Work out the finished part from the listing and answer in its coordinate system (mm). Coordinates: 2 decimals unless noted, no trailing zeros. Loops run counter-clockwise (first coordinate to the right, second up) from the corner with the lowest first, then second, coordinate; pieces in that order, holes last. Notation, with made-up numbers: (88.25, -8.75) -> (145.25, -8.75) arc R18 ccw to (145.25, 9.25) -> close; hole circle Ø9 at (-38.75, 82.5). An arc over 180 degrees is marked (long way). Use a Markdown table: item, result.
from build123d import *

# Parameters (mm, degrees)
SKETCH_1_R          = 38
EXTRUDE_1_DEPTH     = 678
SKETCH_2_R          = 7.5
EXTRUDE_2_DEPTH     = 146.75
SKETCH_3_R          = 8.25
EXTRUDE_4_DEPTH     = 76
EXTRUDE_START       = 76
SKETCH_4_R          = 8.25
EXTRUDE_5_DEPTH     = 76
CUT_EXTRUDE_START   = 7.5
CUT_EXTRUDE_2_DEPTH = 3
SKETCH_9_R          = 14.996083322
CUT_EXTRUDE_4_DEPTH = 34.45


with BuildPart() as part:
    # 草图1 → 凸台-拉伸1 (new, symmetric)
    with BuildSketch(Plane.XY):
        Circle(SKETCH_1_R)
    extrude(amount=EXTRUDE_1_DEPTH, both=True)

    # 草图2 → 凸台-拉伸2 (add, symmetric)
    with BuildSketch(Plane.XY.offset(678)):
        with Locations(Location((0, 0, 0), (0, 0, 180))):
            Circle(SKETCH_2_R)
    extrude_2 = extrude(amount=EXTRUDE_2_DEPTH, both=True)

    # 镜向1: 凸台-拉伸2 across plane
    add(extrude_2.mirror(Plane.XY))

    # 草图3 → 凸台-拉伸4 (add)
    with BuildSketch(Plane.XY.offset(678)):
        Circle(SKETCH_3_R)
    extrude(amount=EXTRUDE_4_DEPTH)

    # 草图4 → 凸台-拉伸5 (add)
    with BuildSketch(Plane(origin=(0, 0, -678), x_dir=(-1, 0, 0), z_dir=(0, 0, -1)).offset(EXTRUDE_START)):
        with Locations(Location((0, 0, 0), (0, 0, 180))):
            Circle(SKETCH_4_R)
    extrude(amount=-EXTRUDE_5_DEPTH)

    # 草图6 → 切除-拉伸2 (cut)
    with BuildSketch(Plane(origin=(0, 0, 0), x_dir=(1, 0, 0), z_dir=(0, 1, 0)).offset(CUT_EXTRUDE_START)):
        with BuildLine():
            Line((-2.5, -824.75), (-2.5, -809.75))
            ThreePointArc((-2.5, -809.75), (0, -807.25), (2.5, -809.75))
            Line((2.5, -809.75), (2.5, -824.75))
            ThreePointArc((2.5, -824.75), (0, -827.25), (-2.5, -824.75))
        make_face()
    cut_extrude_2 = extrude(amount=-CUT_EXTRUDE_2_DEPTH, mode=Mode.SUBTRACT)

    # 镜向2: 切除-拉伸2 across plane
    add(cut_extrude_2.mirror(Plane.XY), mode=Mode.SUBTRACT)

    # 草图9 → 切除-拉伸4 (cut)
    with BuildSketch(Plane.XY.offset(824.75)):
        Circle(SKETCH_9_R)
    extrude(amount=-CUT_EXTRUDE_4_DEPTH, mode=Mode.SUBTRACT)


solid = part.part
Q1. Given pin 1 Ø1 at (y, z) = (-14.5, 232) entering from -X; pin 2 Ø10 at (x, y) = (-27, -24.5) entering from -Z; pin 3 Ø1.5 at (x, z) = (0.5, -819) entering from +Y, each flat-ended and moving along its own axis, determine where each tip first touches the part or whether it passes through.
Solved:
| item | result |
|---|---|
| pin 1 | x = -35.33 |
| pin 2 | z = -678 |
| pin 3 | y = 4.5 |
Q2. Section A-A on z = -340.5 is taken. Determine the outline of the cut face in (x, y).
Solved:
| item | result |
|---|---|
| outline | circle Ø76 at (0, 0) |
Q3. Section B-B on y = 20 is taken. Determine the outline of the cut face in (x, z).
Solved:
| item | result |
|---|---|
| outline | (-32.31, -678) -> (32.31, -678) -> (32.31, 678) -> (-32.31, 678) -> close |
Q4. Consider line 1 (X direction, y = -4, z = 403.5); line 2 (Z direction, x = -26.5, y = 9.5); line 3 (Y direction, x = 0, z = 191). Determine where each line is inside the solid, lowest interval first. Write a range as [from, to].
Solved:
| item | result |
|---|---|
| line 1 | [-37.79, 37.79] |
| line 2 | [-678, 678] |
| line 3 | [-38, 38] |
